Part model, mm, in its own coordinate system. Give positions to 0.01 mm unless a question says otherwise; leave off trailing zeros. Write each loop counter-clockwise with the first axis right and the second up, starting at its lowest first coordinate (ties: lowest second). Pieces come first, ordered by that corner, then holes.
```python
from build123d import *

# Parameters (mm, degrees)
BOSS_EXTRUDE1_DEPTH      = 2
BOSS_EXTRUDE1_DEPTH_BACK = 5
SKETCH1_R                = 13.9
SKETCH2_R                = 3.9
CUT_EXTRUDE1_DEPTH       = 6
SKETCH3_R                = 3.5
BOSS_EXTRUDE2_DEPTH      = 18


with BuildPart() as part:
    # Sketch1 → Boss-Extrude1 (new, two sides: drawn at the far end of the back side and taken through both)
    with BuildSketch(Plane.XY.offset(-BOSS_EXTRUDE1_DEPTH_BACK)):
        with Locations((0.613489308, -35)):
            Circle(SKETCH1_R)
    extrude(amount=BOSS_EXTRUDE1_DEPTH + BOSS_EXTRUDE1_DEPTH_BACK)

    # Sketch2 → Cut-Extrude1 (cut)
    with BuildSketch(Plane(origin=(0, 0, -5), x_dir=(-1, 0, 0), z_dir=(0, 0, -1))):
        with Locations((-0.613489308, -35)):
            Circle(SKETCH2_R)
    extrude(amount=-CUT_EXTRUDE1_DEPTH, mode=Mode.SUBTRACT)

    # Sketch3 → Boss-Extrude2 (add)
    with BuildSketch(Plane.XY.offset(2)):
        with Locations((0.613489308, -42.5)):
            Circle(SKETCH3_R)
    extrude(amount=BOSS_EXTRUDE2_DEPTH)


solid = part.part
```
1) Saw through at B-B, the plane z = 8. Write the cut outline in (x, y), then the cut area to 3 significant figures.
Answers follow:
outline: circle Ø7 at (0.61, -42.5)
area: 38.5 mm2
2) Wall check: L1, parallel to Z at x = 3.5, y = -33.75; L2, parallel to Z at x = 8.25, y = -44.5; L3, parallel to Y at x = -2, z = -3.5. Give the ranges that are in metal, low to high.
Answers follow:
L1: z = 1 to 2
L2: z = -5 to 2
L3: y = -48.65 to -37.89, -32.11 to -21.35
3) Saw through at A-A, the plane y = -35. Write the cut outline in (x, z).
Answers follow:
outline: (-13.29, -5) - (-3.29, -5) - (-3.29, 1) - (4.51, 1) - (4.51, -5) - (14.51, -5) - (14.51, 2) - (-13.29, 2) - close
4) Two-plate mould, pull along Y, no slides. Class faces 1 (the face through (0.16, -39.03, 10.87)), 2 (the face through (1, -35, 1)), 3 (the face through (-1.19, -38.46, -2.04)), 4 (the face through (4, -38, -5)): +Y half, -Y half, draft (parallel to the pull), parting line (faces both ways), or undercut.
Answers follow:
face 1: parting line
face 2: undercut
face 3: undercut
face 4: draft
5) Saw through at C-C, the plane x = 1.5. Write the cut outline in (y, z), then the cut area to 3 significant figures.
Answers follow:
outline: (-48.87, -5) - (-38.8, -5) - (-38.8, 1) - (-31.2, 1) - (-31.2, -5) - (-21.13, -5) - (-21.13, 2) - (-39.11, 2) - (-39.11, 20) - (-45.89, 20) - (-45.89, 2) - (-48.87, 2) - close
area: 271 mm2
6) Saw through at D-D, the plane y = -42.5. Write the cut outline in (x, z).
Answers follow:
outline: (-11.09, -5) - (12.32, -5) - (12.32, 2) - (4.11, 2) - (4.11, 20) - (-2.89, 20) - (-2.89, 2) - (-11.09, 2) - close
7) Pin check, flat tips, straight feed: pin 1 Ø2.5 at (x, y) = (0, -34) entering from -Z; pin 2 Ø14 at (x, y) = (5, -30.5) entering from +Z; pin 3 Ø8 at (x, z) = (-7.5, 3.5) entering from -Y; pin 4 Ø1 at (x, y) = (-10.5, -25.5) entering from -Z (1 decimal). Stop position of each tip, or through.
Answers follow:
pin 1: stops at z = 1
pin 2: stops at z = 2
pin 3: stops at y = -48.18
pin 4: passes through
